The model under review builds one solid part; all positions refer to its coordinate system, in mm. Coordinates: 2 decimals unless noted, no trailing zeros. Order: outer loops, then holes, each group sorted by start corner. A loop starts at its lowest first (then second) coordinate and runs counter-clockwise, first axis right, second up. Notation, with made-up numbers: (23, 62.5) -> (76, 62.5) arc R25 ccw to (76, 79.5) -> close; hole circle Ø6 at (12.5, 6). An arc over 180 degrees is marked (long way). Put each result on its own line as item: value.
from build123d import *

# Parameters (mm, degrees)
BASE_PLATE_PROFILE_WITH_4_HOLES_W = 115
BASE_PLATE_PROFILE_WITH_4_HOLES_H = 40
BASE_PLATE_PROFILE_WITH_4_HOLES_R = 2.5
BASE_PLATE_115X40X5_DEPTH         = 5


with BuildPart() as part:
    # Base Plate Profile with 4 Holes → Base Plate 115x40x5 (new body)
    with BuildSketch(Plane(origin=(0, 0, 0), x_dir=(1, 0, 0), z_dir=(0, 1, 0))):
        Rectangle(BASE_PLATE_PROFILE_WITH_4_HOLES_W, BASE_PLATE_PROFILE_WITH_4_HOLES_H)
        with Locations(Location((-32.5, 10.041360294, 0), (0, 0, 270))):
            Circle(BASE_PLATE_PROFILE_WITH_4_HOLES_R, mode=Mode.SUBTRACT)
        with Locations(Location((-32.5, -9.958639706, 0), (0, 0, 270))):
            Circle(BASE_PLATE_PROFILE_WITH_4_HOLES_R, mode=Mode.SUBTRACT)
        with Locations(Location((32.5, -9.958639706, 0), (0, 0, 90))):
            Circle(BASE_PLATE_PROFILE_WITH_4_HOLES_R, mode=Mode.SUBTRACT)
        with Locations(Location((32.5, 10.041360294, 0), (0, 0, 90))):
            Circle(BASE_PLATE_PROFILE_WITH_4_HOLES_R, mode=Mode.SUBTRACT)
    extrude(amount=BASE_PLATE_115X40X5_DEPTH)


solid = part.part
Item 1: Consider section C-C on z = 10. Write out the cut boundary in (x, y).
Answers below:
outline: (-57.5, 0) -> (-35, 0) -> (-35, 5) -> (-57.5, 5) -> close; (-30, 0) -> (30, 0) -> (30, 5) -> (-30, 5) -> close; (35, 0) -> (57.5, 0) -> (57.5, 5) -> (35, 5) -> close
Item 2: Consider section B-B on y = 1.65. Write out the cut boundary in (x, z), and give its area (3 significant figures).
Answers below:
outline: (-57.5, -20) -> (57.5, -20) -> (57.5, 20) -> (-57.5, 20) -> close; hole circle Ø5 at (-32.5, -10.04); hole circle Ø5 at (-32.5, 9.96); hole circle Ø5 at (32.5, -10.04); hole circle Ø5 at (32.5, 9.96)
area: 4,520 mm^2
Item 3: Consider section A-A on x = 32.5. Write out the cut boundary in (y, z), and give its area (3 significant figures).
Answers below:
outline: (0, -20) -> (5, -20) -> (5, -12.54) -> (0, -12.54) -> close; (0, -7.54) -> (5, -7.54) -> (5, 7.46) -> (0, 7.46) -> close; (0, 12.46) -> (5, 12.46) -> (5, 20) -> (0, 20) -> close
area: 150 mm^2
Item 4: Mouldability with a two-part tool opening along X and no side actions: class faces 1 (the cylindrical face through (30, 2, -10)), 2 (the flat face through (-57.5, 2, 0)), 3 (the flat face through (-1, 2, -20)), 4 (the flat face through (57.5, 2, 0)) as +X half, -X half, draft (parallel to the pull), parting line (faces both ways), or undercut.
Answers below:
face 1: undercut
face 2: -X half
face 3: draft
face 4: +X half
Item 5: For line 1 (Z direction, x = 32.5, y = 3.95); line 2 (X direction, y = 2.4, z = -11.5); line 3 (Z direction, x = 31.5, y = 1.1), list the stretches that pass through material, from the lowest coordinate up. Write a range as from..to.
Answers below:
line 1: -20..-12.54, -7.54..7.46, 12.46..20
line 2: -57.5..-34.53, -30.47..30.47, 34.53..57.5
line 3: -20..-12.33, -7.75..7.67, 12.25..20
Item 6: For pin 1 Ø8 at (x, z) = (32.5, 9.96) entering from +Y, flat-tipped, find the tip position at first contact; note if it passes through.
Answers below:
pin 1: y = 5
